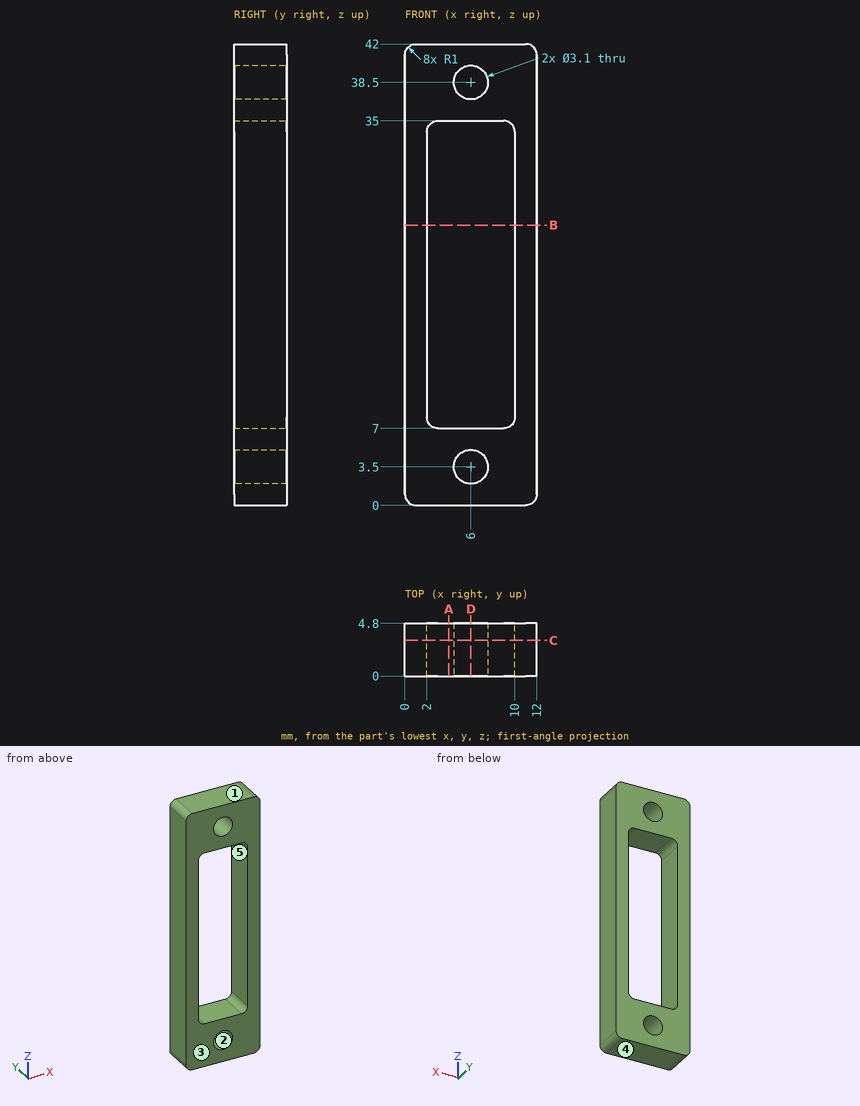
For this review, use the dimensioned drawing (mm, ordinates from the lowest corner) and the shaded views. A direction names the side the tool comes from. Round coordinates to 2 decimals unless told otherwise and drop trailing zeros. Order: outer loops, then holes, each group sorted by start corner. A loop starts at its lowest first (then second) coordinate and runs counter-clockwise, first axis right, second up. Notation, with made-up numbers: M 15,41 L 69,41 A22 ccw 69,73 Z; hole C 22,58.25 d6. An arc over 180 degrees is marked long. Write each question's results on one line, items separated by ' | '. Start each with the question number.
1. Draft analysis for pull direction Z (two halves, no side actions). For the marked faces 1, 2 and 3, state which applies: pulls with the +Z half, pulls with the -Z half, needs draft (parallel to the pull), parting line crosses it, or undercut.
2. Tool access review of the marked faces 4 and 5: name each direction out of +Z, -Z, +X, -X, +Y, -Y from which nothing blocks a thin tool from reaching the whole face with its end or side.
3. To check wall thickness, follow L1, parallel to X at y = 1.65, z = 3.5; L2, parallel to Z at x = 3.25, y = 2.6; L3, parallel to X at y = 0.9, z = 21.5. State the ranges of each line that lie inside material, in increasing order. Write a range as [from, to].
4. Add section C-C (y = 3.25). State the section outline as (x, z) points.
5. Add section D-D (x = 6). State the section outline as (y, z) points, then the cut area to 3 significant figures.
6. Add section B-B (z = 25.5). State the section outline as (x, y) points.
7. Add section A-A (x = 4). State the section outline as (y, z) points.
Output values:
1) face 1: pulls with the +Z half | face 2: undercut | face 3: needs draft
2) face 4: -Z, +X, -X, +Y, -Y | face 5: +Y, -Y
3) L1: [0, 4.45], [7.55, 12] | L2: [0, 7], [35, 42] | L3: [0, 2], [10, 12]
4) outline: M 0,1 A1 ccw 1,0 L 11,0 A1 ccw 12,1 L 12,41 A1 ccw 11,42 L 1,42 A1 ccw 0,41 Z; hole M 2,8 A1 ccw 3,7 L 9,7 A1 ccw 10,8 L 10,34 A1 ccw 9,35 L 3,35 A1 ccw 2,34 Z; hole C 6,3.5 d3.1; hole C 6,38.5 d3.1
5) outline: M 0,0 L 4.8,0 L 4.8,1.95 L 0,1.95 Z; M 0,5.05 L 4.8,5.05 L 4.8,7 L 0,7 Z; M 0,35 L 4.8,35 L 4.8,36.95 L 0,36.95 Z; M 0,40.05 L 4.8,40.05 L 4.8,42 L 0,42 Z | area: 37.4 mm^2
6) outline: M 0,0 L 2,0 L 2,4.8 L 0,4.8 Z; M 10,0 L 12,0 L 12,4.8 L 10,4.8 Z
7) outline: M 0,0 L 4.8,0 L 4.8,7 L 0,7 Z; M 0,35 L 4.8,35 L 4.8,42 L 0,42 Z
